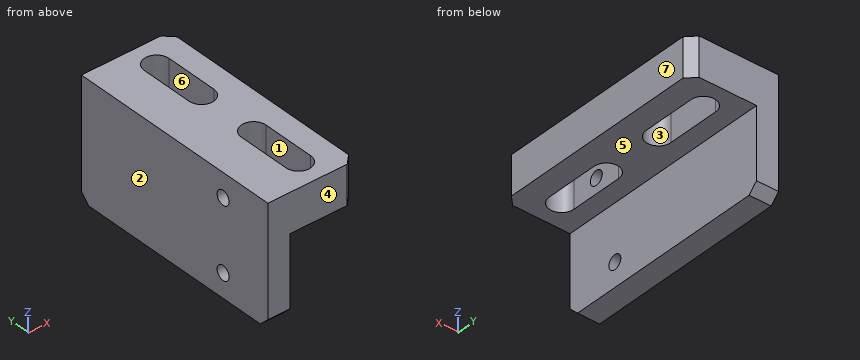
from build123d import *

# Parameters (mm, degrees)
SKETCH1_W             = 10
SKETCH1_H             = 13.4
BOSS_EXTRUDE1_DEPTH   = 25
CUT_EXTRUDE2_DEPTH    = 14
M2_TAPPED_HOLE1_D     = 1.6
M2_TAPPED_HOLE1_DEPTH = 5.2
M2_TAPPED_HOLE1_TIP   = 0.480688495
SKETCH7_W             = 9.563839575
SKETCH7_H             = 25
CUT_EXTRUDE3_DEPTH    = 9
CHAMFER1_SIZE         = 1


with BuildPart() as part:
    # Sketch1 → Boss-Extrude1 (new body)
    with BuildSketch(Plane(origin=(0, 0, 0), x_dir=(1, 0, 0), z_dir=(0, 1, 0))):
        with Locations((5, 6.7)):
            Rectangle(SKETCH1_W, SKETCH1_H)
    extrude(amount=BOSS_EXTRUDE1_DEPTH)

    # Q → Cut-Extrude2 (cut)
    with BuildSketch(Plane.XY):
        with BuildLine():
            Line((7.4, 22), (7.4, 16))
            ThreePointArc((7.4, 16), (6, 14.6), (4.6, 16))
            Line((4.6, 16), (4.6, 22))
            ThreePointArc((4.6, 22), (6, 23.4), (7.4, 22))
        make_face()
        with BuildLine():
            Line((7.4, 3), (7.4, 9))
            ThreePointArc((7.4, 9), (6, 10.4), (4.6, 9))
            Line((4.6, 9), (4.6, 3))
            ThreePointArc((4.6, 3), (6, 1.6), (7.4, 3))
        make_face()
    extrude(amount=-CUT_EXTRUDE2_DEPTH, mode=Mode.SUBTRACT)

    # M2 Tapped Hole1
    with Locations(Plane.ZY):
        with Locations((-10.7, 6), (-2.7, 6)):
            Hole(M2_TAPPED_HOLE1_D / 2, depth=M2_TAPPED_HOLE1_DEPTH)
            with Locations((0, 0, -(M2_TAPPED_HOLE1_DEPTH + M2_TAPPED_HOLE1_TIP / 2))):  # 118° drill point
                Cone(0, M2_TAPPED_HOLE1_D / 2, M2_TAPPED_HOLE1_TIP, mode=Mode.SUBTRACT)

    # Sketch7 → Cut-Extrude3 (cut)
    with BuildSketch(Plane(origin=(0, 0, -13.4), x_dir=(-1, 0, 0), z_dir=(0, 0, -1))):
        with Locations((-7.281919788, 12.5)):
            Rectangle(SKETCH7_W, SKETCH7_H)
    extrude(amount=-CUT_EXTRUDE3_DEPTH, mode=Mode.SUBTRACT)

    # Chamfer1
    chamfer1_edges = [part.edges().sort_by_distance(p)[0] for p in [
        (10, 25, -2.2),
        (10, 0, -2.2),
        (1.25, 0, -13.4),
        (1.25, 25, -13.4),
    ]]
    chamfer(chamfer1_edges, length=CHAMFER1_SIZE)


solid = part.part
Could you check a few things on this model? Use its own coordinates, in mm. Face numbers are marked on the shaded views. A direction names the side the tool comes from. Round coordinates to 2 decimals unless told otherwise and drop trailing zeros. Write each loop counter-clockwise with the first axis right and the second up, starting at its lowest first coordinate (ties: lowest second). Pieces come first, ordered by that corner, then holes. Notation, with made-up numbers: (-26.5, -2) -> (2.5, -2) arc R24 ccw to (2.5, 31) -> close; hole circle Ø3 at (-35.75, 52). An arc over 180 degrees is marked (long way). Use a Markdown table: item, result.
1. If we section it at B-B (z = -10.7): List the corners of the cut face in (x, y) for me, then the cut area to 3 significant figures.
Answer key:
| item | result |
|---|---|
| outline | (0, 0) -> (2.5, 0) -> (2.5, 5.2) -> (0, 5.2) -> close; (0, 6.8) -> (2.5, 6.8) -> (2.5, 25) -> (0, 25) -> close |
| area | 58.5 mm^2 |
2. If we section it at A-A (y = 6): List the corners of the cut face in (x, z) for me, then the cut area to 3 significant figures.
Answer key:
| item | result |
|---|---|
| outline | (0, -13.4) -> (2.5, -13.4) -> (2.5, -11.5) -> (0, -11.5) -> close; (0, -9.9) -> (2.5, -9.9) -> (2.5, -4.4) -> (4.6, -4.4) -> (4.6, -3.5) -> (0, -3.5) -> close; (0, -1.9) -> (4.6, -1.9) -> (4.6, 0) -> (0, 0) -> close; (7.4, -4.4) -> (10, -4.4) -> (10, 0) -> (7.4, 0) -> close |
| area | 42.8 mm^2 |
3. For pin 1 Ø3 at (x, y) = (4.5, 14) entering from -Z; pin 2 Ø8 at (y, z) = (13.5, -8.5) entering from +X; pin 3 Ø1.8 at (y, z) = (6, -10.7) entering from -X; pin 4 Ø4 at (x, z) = (5.5, -8) entering from +Y, each with a flat end and sliding along its axis, tell me the tip position at first contact or that it passes through.
Answer key:
| item | result |
|---|---|
| pin 1 | stops at z = -4.4 |
| pin 2 | stops at x = 2.5 |
| pin 3 | stops at x = 0 |
| pin 4 | passes through |
4. Please list where these lines run through material, in increasing order: probe 1 along Y at (x, z) = (4.75, -2.75); probe 2 along X at (y, z) = (20, -0.75); probe 3 along Y at (x, z) = (1.7, -10.7).
Answer key:
| item | result |
|---|---|
| probe 1 | y = 0 to 2.37, 9.63 to 15.37, 22.63 to 25 |
| probe 2 | x = 0 to 4.6, 7.4 to 10 |
| probe 3 | y = 0 to 5.2, 6.8 to 25 |
5. Which directions (+Z, -Z, +X, -X, +Y, -Y) give clear straight access to the entire face, cutting with the end or side of a thin tool? Please do the marked faces 5, 6 and 7.
Answer key:
| item | result |
|---|---|
| face 5 | -Z, +X, +Y, -Y |
| face 6 | +Z, -Z |
| face 7 | +Z, -Z, +X, +Y, -Y |
6. If we section it at D-D (z = -1.5): List the corners of the cut face in (x, y) for me.
Answer key:
| item | result |
|---|---|
| outline | (0, 0) -> (9, 0) -> (10, 1) -> (10, 24) -> (9, 25) -> (0, 25) -> close; hole (4.6, 3) arc R1.4 ccw to (7.4, 3) -> (7.4, 9) arc R1.4 ccw to (4.6, 9) -> close; hole (4.6, 16) arc R1.4 ccw to (7.4, 16) -> (7.4, 22) arc R1.4 ccw to (4.6, 22) -> close |
7. If we section it at C-C (x = 6): List the corners of the cut face in (y, z) for me.
Answer key:
| item | result |
|---|---|
| outline | (0, -4.4) -> (1.6, -4.4) -> (1.6, 0) -> (0, 0) -> close; (10.4, -4.4) -> (14.6, -4.4) -> (14.6, 0) -> (10.4, 0) -> close; (23.4, -4.4) -> (25, -4.4) -> (25, 0) -> (23.4, 0) -> close |
8. We'd pull the mould along X, two halves only. Please class the marked faces 1, 2, 3 and 4: +X half, -X half, draft (parallel to the pull), parting line (faces both ways), or undercut.
Answer key:
| item | result |
|---|---|
| face 1 | undercut |
| face 2 | -X half |
| face 3 | undercut |
| face 4 | draft |
